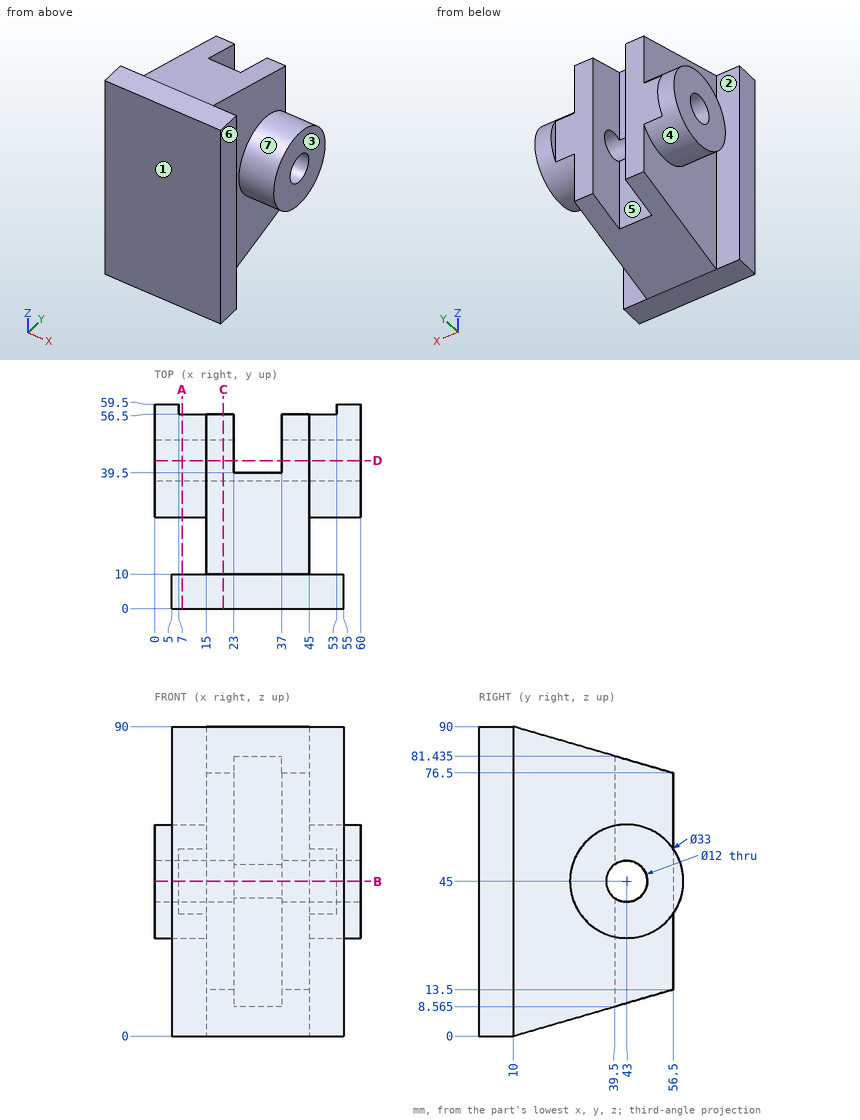
Study the drawing (mm; zero at the part's minimum x, y, z) and answer. A direction names the side the tool comes from. Round coordinates to 2 decimals unless told otherwise and drop trailing zeros. Loops run counter-clockwise (first coordinate to the right, second up) from the corner with the lowest first, then second, coordinate; pieces in that order, holes last. Notation, with made-up numbers: (39, 82) -> (63, 82) arc R12 cw to (63, 100) -> close; hole circle Ø6 at (74, -27.75). An arc over 180 degrees is marked (long way). Use one line per item in the form item = value.
1. The part is cut by section C-C on x = 20. Determine the outline of the cut face in (y, z), and give its area (3 significant figures).
Answer key:
outline = (0, 0) -> (10, 0) -> (56.5, 13.5) -> (56.5, 76.5) -> (10, 90) -> (0, 90) -> close; hole circle Ø12 at (43, 45)
area = 4,340 mm²
2. The part is cut by section B-B on z = 45. Determine the outline of the cut face in (x, y), and give its area (3 significant figures).
Answer key:
outline = (0, 26.5) -> (15, 26.5) -> (15, 10) -> (5, 10) -> (5, 0) -> (55, 0) -> (55, 10) -> (45, 10) -> (45, 26.5) -> (60, 26.5) -> (60, 37) -> (0, 37) -> close; (0, 49) -> (23, 49) -> (23, 56.5) -> (7, 56.5) -> (7, 59.5) -> (0, 59.5) -> close; (37, 49) -> (60, 49) -> (60, 59.5) -> (53, 59.5) -> (53, 56.5) -> (37, 56.5) -> close
area = 2,010 mm²
3. For a pull along Y with two mould halves and no side action, classify the marked faces 1, 2 and 3 as released by +Y, released by -Y, zero draft, split by the parting line, or undercut.
Answer key:
face_1 = released by -Y
face_2 = undercut
face_3 = zero draft
4. The part is cut by section A-A on x = 8. Determine the outline of the cut face in (y, z).
Answer key:
outline = (0, 0) -> (10, 0) -> (10, 90) -> (0, 90) -> close; (56.5, 35.51) -> (56.5, 54.49) arc R16.5 ccw (long way) to start; hole circle Ø12 at (43, 45)
5. Flat-ended cylindrical pins translate along their axes: pin 1 Ø3 at (x, y) = (44.5, 22.5) entering from -Z; pin 2 Ø3 at (y, z) = (3, 50) entering from +X; pin 3 Ø10 at (y, z) = (18, 79.5) entering from -X. Find the tip coordinate at first contact, or state that the pin passes through.
Answer key:
pin_1 = 3.19
pin_2 = 55
pin_3 = 15
6. Find the intervals of material crossed by probe 1 along Y at (x, z) = (14, 45); probe 2 along Y at (x, z) = (16, 45); probe 3 along X at (y, z) = (46.5, 63.5), in increasing order. Write a range as [from, to].
Answer key:
probe_1 = [0, 10], [26.5, 37], [49, 56.5]
probe_2 = [0, 37], [49, 56.5]
probe_3 = [15, 23], [37, 45]
7. The part is cut by section D-D on y = 43. Determine the outline of the cut face in (x, z).
Answer key:
outline = (0, 28.5) -> (15, 28.5) -> (15, 9.58) -> (23, 9.58) -> (23, 39) -> (0, 39) -> close; (0, 51) -> (23, 51) -> (23, 80.42) -> (15, 80.42) -> (15, 61.5) -> (0, 61.5) -> close; (37, 9.58) -> (45, 9.58) -> (45, 28.5) -> (60, 28.5) -> (60, 39) -> (37, 39) -> close; (37, 51) -> (60, 51) -> (60, 61.5) -> (45, 61.5) -> (45, 80.42) -> (37, 80.42) -> close
8. A tool of negligible diameter and unlimited length cuts with its end or side. For the marked faces 4, 5, 6 and 7, from which of +Z, -Z, +X, -X, +Y, -Y can it reach the whole face along a straight path? Write none if from no direction.
Answer key:
face_4 = -X
face_5 = +Z, -Z, +Y
face_6 = +Z, -Z, +X, -Y
face_7 = +X
